CAD build for the part. Positions are in the model's coordinates, mm. Face numbers are marked on the shaded views. A direction names the side the tool comes from. Coordinates: 2 decimals unless noted, no trailing zeros. Loops run counter-clockwise (first coordinate to the right, second up) from the corner with the lowest first, then second, coordinate; pieces in that order, holes last. Notation, with made-up numbers: (-2, -15) -> (53, -15) arc R26 cw to (53, 10) -> close; hole circle Ø4 at (88, 38). An arc over 180 degrees is marked (long way). Answer as CSV lines item,"result". Start each with the question number.
```python
from build123d import *

# Parameters (mm, degrees)
SKETCH1_W           = 500
SKETCH1_H           = 500
BOSS_EXTRUDE1_DEPTH = 900
SKETCH2_R           = 150
BOSS_EXTRUDE2_DEPTH = 136
SKETCH3_W           = 1400
SKETCH3_H           = 300
CUT_EXTRUDE1_DEPTH  = 1100.543541657


with BuildPart() as part:
    # Sketch1 → Boss-Extrude1 (new, symmetric)
    with BuildSketch(Plane.XY):
        Rectangle(SKETCH1_W, SKETCH1_H)
    extrude(amount=BOSS_EXTRUDE1_DEPTH, both=True)

    # Sketch2 → Boss-Extrude2 (add)
    with BuildSketch(Plane.XZ.offset(250)):
        with Locations(Location((0, -700, 0), (0, 0, 90))):
            Circle(SKETCH2_R)
        with Locations(Location((0, 700, 0), (0, 0, 90))):
            Circle(SKETCH2_R)
    extrude(amount=BOSS_EXTRUDE2_DEPTH)

    # Sketch3 → Cut-Extrude1 (cut, through all)
    with BuildSketch(Plane(origin=(250, 0, 0), x_dir=(0, 0, -1), z_dir=(1, 0, 0))):
        with Locations((0, 100)):
            Rectangle(SKETCH3_W, SKETCH3_H)
    extrude(amount=-CUT_EXTRUDE1_DEPTH, mode=Mode.SUBTRACT)


solid = part.part
```
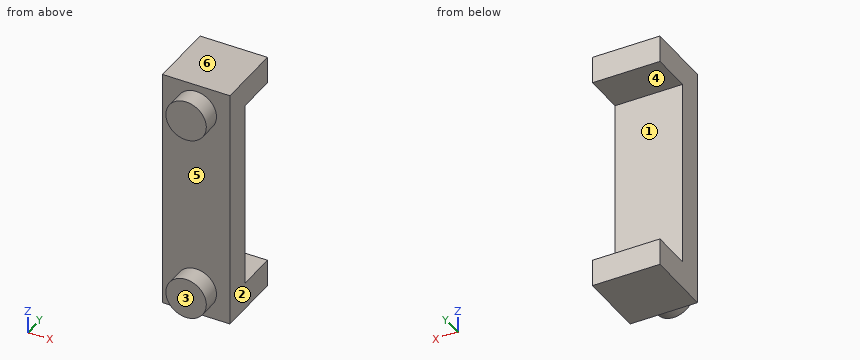
Q1. Saw through at B-B (x = 0). List the corners of the cut face in (y, z).
Q2. Saw through at C-C (z = -736.5). List the corners of the cut face in (x, y), and give its area (3 significant figures).
Q3. Two-plate mould, pull along Z, no slides. Class the marked faces 3, 4, 5 and 6: pulls with the +Z half, pulls with the -Z half, needs draft (parallel to the pull), parting line crosses it, or undercut.
Q4. Which spindle directions (+Z, -Z, +X, -X, +Y, -Y) get a long thin tool onto all of the face, cutting with end or side? Do the marked faces 1 and 2. Say none if no direction does.
Q5. Saw through at D-D (y = -278). List the corners of the cut face in (x, z).
Q6. Saw through at A-A (y = 36). List the corners of the cut face in (x, z), and give its area (3 significant figures).
Q7. Probe probe 1 along Z at (x, y) = (194.5, 217.5); probe 2 along Y at (x, z) = (-147, 616); probe 3 along Y at (x, z) = (138.5, 685). List the from-to ranges inside material, lowest first. Write a range as from..to.
Q8. Pin check, flat tips, straight feed: pin 1 Ø4 at (x, z) = (113, 318) entering from -Y; pin 2 Ø1 at (x, z) = (147.5, -27.5) entering from +Y. Stop position of each tip, or through.
Ans:
1,outline,"(-386, -850) -> (-250, -850) -> (-250, -900) -> (250, -900) -> (250, -700) -> (-50, -700) -> (-50, 700) -> (250, 700) -> (250, 900) -> (-250, 900) -> (-250, 850) -> (-386, 850) -> (-386, 550) -> (-250, 550) -> (-250, -550) -> (-386, -550) -> close"
2,outline,"(-250, -250) -> (-145.49, -250) -> (-145.49, -386) -> (145.49, -386) -> (145.49, -250) -> (250, -250) -> (250, 250) -> (-250, 250) -> close"
2,area,"290,000 mm²"
3,face 3,"needs draft"
3,face 4,"undercut"
3,face 5,"undercut"
3,face 6,"pulls with the +Z half"
4,face 1,"+X, -X, +Y"
4,face 2,"+Z, -Z, +X, +Y, -Y"
5,outline,"circle Ø300 at (0, -700); circle Ø300 at (0, 700)"
6,outline,"(-250, -900) -> (250, -900) -> (250, -700) -> (-250, -700) -> close; (-250, 700) -> (250, 700) -> (250, 900) -> (-250, 900) -> close"
6,area,"200,000 mm²"
7,probe 1,"z = -900..-700, 700..900"
7,probe 2,"y = -250..-50"
7,probe 3,"y = -386..-50"
8,pin 1,"stops at y = -250"
8,pin 2,"stops at y = -50"
